Source: CAD feature listing. Evaluate the final solid. Frame: model axes, mm. Coordinates: 2 decimals unless noted, no trailing zeros. Write each loop counter-clockwise with the first axis right and the second up, starting at its lowest first coordinate (ties: lowest second). Pieces come first, ordered by that corner, then holes. Notation, with made-up numbers: M 8,-35 L 51,-35 A26 cw 51,-15 Z; hole C 17.25,29 d7. An arc over 180 degrees is marked long. One line per item, written item: value. Start each with the question number.
Item 1: Ray query, L1, parallel to X at y = 158.75, z = 0; L2, parallel to X at y = 17, z = 5.25; L3, parallel to X at y = -71, z = -0.25. Return the intervals inside material, ascending. Write a range as from..to.
Item 2: Pin query (flat end, axial travel): P1, Ø1.5, axis at x = -3.5, y = 42.5, coming from the +Z side; P2, Ø4.5, axis at x = 0, z = 0, coming from the -Y side; P3, Ø2.5, axis at y = -134.5, z = -1.5, coming from the +X side. Return the tip coordinate at first contact, or that it passes through.
Item 3: Cut plane A-A, the plane y = 22.5. Output: boundary loops of the cut face in (x, z), then the cut area to 3 significant figures.
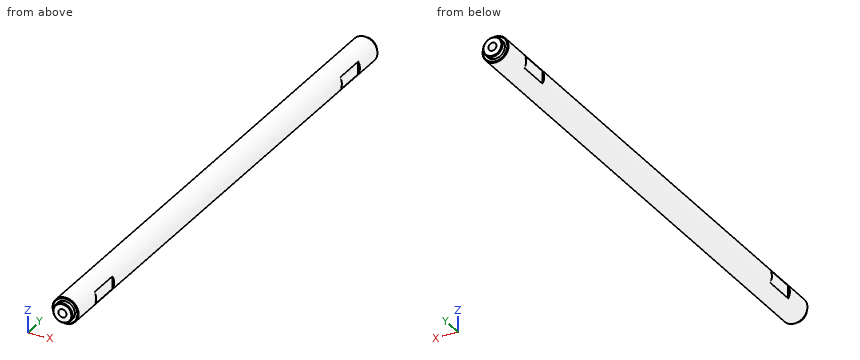
```python
from build123d import *

# Parameters (mm, degrees)
SKETCH1_R             = 8
BOSS_EXTRUDE1_DEPTH   = 166.5
SKETCH2_R             = 6
BOSS_EXTRUDE2_DEPTH   = 3
CHAMFER1_SIZE         = 0.5
CUT_EXTRUDE2_START    = -40
CUT_EXTRUDE2_DEPTH    = 20
M6_TAPPED_HOLE1_D     = 5
M6_TAPPED_HOLE1_DEPTH = 17
M6_TAPPED_HOLE1_TIP   = 1.502151548
CHAMFER2_SIZE         = 0.5
BOSS_EXTRUDE3_START   = 3
SKETCH6_R             = 6
BOSS_EXTRUDE3_DEPTH   = 3
CHAMFER3_SIZE         = 0.5
M6_TAPPED_HOLE2_D     = 5
M6_TAPPED_HOLE2_DEPTH = 17
M6_TAPPED_HOLE2_TIP   = 1.502151548


with BuildPart() as part:
    # Sketch1 → Boss-Extrude1 (new, symmetric)
    with BuildSketch(Plane(origin=(0, 0, 0), x_dir=(1, 0, 0), z_dir=(0, 1, 0))):
        with Locations(Location((0, 0, 0), (0, 0, 270))):
            Circle(SKETCH1_R)
    extrude(amount=BOSS_EXTRUDE1_DEPTH, both=True)

    # Sketch2 → Boss-Extrude2 (add)
    with BuildSketch(Plane.XZ.offset(166.5)):
        with Locations(Location((0, 0, 0), (0, 0, 90))):
            Circle(SKETCH2_R)
    extrude(amount=BOSS_EXTRUDE2_DEPTH)

    # Chamfer1
    chamfer1_edges = [part.edges().sort_by_distance(p)[0] for p in [
        (0, -166.5, -8),
        (0, -169.5, -6),
    ]]
    chamfer(chamfer1_edges, length=CHAMFER1_SIZE)

    # Sketch3 → Cut-Extrude2 (cut)
    with BuildSketch(Plane.XZ.offset(166.5).offset(CUT_EXTRUDE2_START)):
        with BuildLine():
            Line((-7, 3.872983346), (-7, -3.872983346))
            ThreePointArc((-7, -3.872983346), (-8, 0), (-7, 3.872983346))
        make_face()
        with BuildLine():
            Line((7, 3.872983346), (7, -3.872983346))
            ThreePointArc((7, -3.872983346), (8, 0), (7, 3.872983346))
        make_face()
    cut_extrude2 = extrude(amount=CUT_EXTRUDE2_DEPTH, mode=Mode.SUBTRACT)

    # M6 Tapped Hole1
    with Locations(Plane.XZ.offset(169.5)):
        with Locations((0, 0)):
            Hole(M6_TAPPED_HOLE1_D / 2, depth=M6_TAPPED_HOLE1_DEPTH)
            with Locations((0, 0, -(M6_TAPPED_HOLE1_DEPTH + M6_TAPPED_HOLE1_TIP / 2))):  # 118° drill point
                Cone(0, M6_TAPPED_HOLE1_D / 2, M6_TAPPED_HOLE1_TIP, mode=Mode.SUBTRACT)

    # Chamfer2
    chamfer2_edges = [part.edges().sort_by_distance(p)[0] for p in [
        (0, 166.5, -8),
    ]]
    chamfer(chamfer2_edges, length=CHAMFER2_SIZE)

    # Sketch6 → Boss-Extrude3 (add)
    with BuildSketch(Plane(origin=(0, 166.5, 0), x_dir=(1, 0, 0), z_dir=(0, 1, 0)).offset(BOSS_EXTRUDE3_START)):
        with Locations(Location((0, 0, 0), (0, 0, 270))):
            Circle(SKETCH6_R)
    extrude(amount=-BOSS_EXTRUDE3_DEPTH)

    # Chamfer3
    chamfer3_edges = [part.edges().sort_by_distance(p)[0] for p in [
        (0, 169.5, -6),
    ]]
    chamfer(chamfer3_edges, length=CHAMFER3_SIZE)

    # M6 Tapped Hole2
    with Locations(Plane(origin=(0, 169.5, 0), x_dir=(-1, 0, 0), z_dir=(0, 1, 0))):
        with Locations((0, 0)):
            Hole(M6_TAPPED_HOLE2_D / 2, depth=M6_TAPPED_HOLE2_DEPTH)
            with Locations((0, 0, -(M6_TAPPED_HOLE2_DEPTH + M6_TAPPED_HOLE2_TIP / 2))):  # 118° drill point
                Cone(0, M6_TAPPED_HOLE2_D / 2, M6_TAPPED_HOLE2_TIP, mode=Mode.SUBTRACT)

    # Mirror1: Cut-Extrude2 across plane
    add(cut_extrude2.mirror(Plane.ZX), mode=Mode.SUBTRACT)


solid = part.part
```
From the geometry:
1. L1: x = -8..-2.5, 2.5..8
1. L2: x = -6.04..6.04
1. L3: x = -8..8
2. P1: stops at z = 7.51
2. P2: stops at y = -152.35
2. P3: stops at x = 7
3. outline: C 0,0 d16
3. area: 201 mm²
